Could you check a few things on this model? Use its own coordinates, in mm. Coordinates: 2 decimals unless noted, no trailing zeros. Loops run counter-clockwise (first coordinate to the right, second up) from the corner with the lowest first, then second, coordinate; pieces in that order, holes last.
1) Will these pins go through, and if not, where does the flat tip stop? P1, Ø1.5, axis at y = 7, z = -24.5, coming from the +X side; P2, Ø1, axis at y = 7.5, z = -3, coming from the +X side; P3, Ø2, axis at y = 1.5, z = 5.5, coming from the -X side.
2) Thinking about a two-plate mould opening in X: for faces 1 (the face through (-29.775, 4.944, -6.612)), 2 (the face through (-11, 0, -30)), 3 (the face through (-22.818, 4.944, -29.759)), which applies, released by +X, released by -X, zero draft, split by the parting line, or undercut?
3) Imagine slicing it at A-A on z = 0. Please give me the cut outline in (x, y).
4) If I drill on line 1 along X through (y, z) = (3.5, 0); line 2 along Z through (x, y) = (19.5, 1.5); line 3 along Z through (x, y) = (-16, 1.5), over which ranges is the centre line in solid material (lowest first)?
5) Imagine slicing it at C-C on y = 6. Please give me the cut outline in (x, z), plus the area to 3 significant figures.
6) Imagine slicing it at B-B on x = 0. Please give me the cut outline in (y, z).
```python
from build123d import *

# Parameters (mm, degrees)
SKETCH1_R           = 37.5
SKETCH1_R_2         = 30.5
BOSS_EXTRUDE1_DEPTH = 10
CHAMFER1_SIZE       = 1


with BuildPart() as part:
    # Sketch1 → Boss-Extrude1 (new body)
    with BuildSketch(Plane(origin=(0, 0, 0), x_dir=(1, 0, 0), z_dir=(0, 1, 0))):
        with Locations(Location((0, 0, 0), (0, 0, 270))):
            Circle(SKETCH1_R)
        with Locations(Location((0, 0, 0), (0, 0, 270))):
            Circle(SKETCH1_R_2, mode=Mode.SUBTRACT)
    extrude(amount=BOSS_EXTRUDE1_DEPTH)

    # Chamfer1
    chamfer1_edges = [part.edges().sort_by_distance(p)[0] for p in [
        (0, 0, -37.5),
        (0, 10, -37.5),
        (0, 0, -30.5),
        (0, 10, -30.5),
    ]]
    chamfer(chamfer1_edges, length=CHAMFER1_SIZE)


solid = part.part
```
Filled in:
1. P1: stops at x = 29.02
1. P2: stops at x = 37.42
1. P3: stops at x = -37.23
2. face 1: undercut
2. face 2: zero draft
2. face 3: split by the parting line
3. outline: (-37.5, 1) - (-36.5, 0) - (-31.5, 0) - (-30.5, 1) - (-30.5, 9) - (-31.5, 10) - (-36.5, 10) - (-37.5, 9) - close; (30.5, 1) - (31.5, 0) - (36.5, 0) - (37.5, 1) - (37.5, 9) - (36.5, 10) - (31.5, 10) - (30.5, 9) - close
4. line 1: x = -37.5 to -30.5, 30.5 to 37.5
4. line 2: z = -32.03 to -23.45, 23.45 to 32.03
4. line 3: z = -33.92 to -25.97, 25.97 to 33.92
5. outline: circle Ø75 at (0, 0); hole circle Ø61 at (0, 0)
5. area: 1,500 mm2
6. outline: (0, -36.5) - (1, -37.5) - (9, -37.5) - (10, -36.5) - (10, -31.5) - (9, -30.5) - (1, -30.5) - (0, -31.5) - close; (0, 31.5) - (1, 30.5) - (9, 30.5) - (10, 31.5) - (10, 36.5) - (9, 37.5) - (1, 37.5) - (0, 36.5) - close
